```python
from build123d import *
from OCP.BRepFilletAPI import BRepFilletAPI_MakeChamfer

# Parameters (mm, degrees)
SKETCH_1_R          = 5
EXTRUDE_1_DEPTH     = 6
CUT_EXTRUDE_1_DEPTH = 3
SKETCH_3_R          = 3
EXTRUDE_2_DEPTH     = 8
CHAMFER_1_SIZE      = 0.75
FILLET_1_R          = 0.769230769
CHAMFER_2_SIZE      = 1.44092219
CHAMFER_2_SIZE2     = 2.495750443
FILLET_2_R          = 0.1


with BuildPart() as part:
    # 草图1 → 凸台-拉伸1 (new body)
    with BuildSketch(Plane.XY):
        Circle(SKETCH_1_R)
    extrude(amount=EXTRUDE_1_DEPTH)

    # 草图2 → 切除-拉伸1 (cut)
    with BuildSketch(Plane.XY.offset(6)):
        Polygon((2.5, 1.443375673), (0, 2.886751346), (-2.5, 1.443375673), (-2.5, -1.443375673), (0, -2.886751346), (2.5, -1.443375673), align=None)
    extrude(amount=-CUT_EXTRUDE_1_DEPTH, mode=Mode.SUBTRACT)

    # 草图3 → 凸台-拉伸2 (add)
    with BuildSketch(Plane(origin=(0, 0, 0), x_dir=(-1, 0, 0), z_dir=(0, 0, -1))):
        with Locations(Location((0, 0, 0), (0, 0, 180))):
            Circle(SKETCH_3_R)
    extrude(amount=EXTRUDE_2_DEPTH)

    # 倒角1
    chamfer_1_edges = [part.edges().sort_by_distance(p)[0] for p in [
        (-3, 0, -8),
    ]]
    chamfer(chamfer_1_edges, length=CHAMFER_1_SIZE)

    # 圆角1
    fillet_1_edges = [part.edges().sort_by_distance(p)[0] for p in [
        (-5, 0, 6),
    ]]
    fillet(fillet_1_edges, radius=FILLET_1_R)

    # 倒角2: one chamfer whose edges measure the first distance from different faces: ONE call of the kernel's chamfer builder (chamfer() names one face for all edges)
    chamfer_2_edges_1 = [part.edges().sort_by_distance(p)[0] for p in [
        (1.25, 2.165063509, 3),
    ]]
    chamfer_2_side_1 = [part.faces().sort_by_distance(p)[0] for p in [
        (1.25, 2.165063509, 4.5),
    ]]
    chamfer_2_edges_2 = [part.edges().sort_by_distance(p)[0] for p in [
        (2.5, 0, 3),
    ]]
    chamfer_2_side_2 = [part.faces().sort_by_distance(p)[0] for p in [
        (2.5, 0, 4.5),
    ]]
    chamfer_2_edges_3 = [part.edges().sort_by_distance(p)[0] for p in [
        (1.25, -2.165063509, 3),
    ]]
    chamfer_2_side_3 = [part.faces().sort_by_distance(p)[0] for p in [
        (1.25, -2.165063509, 4.5),
    ]]
    chamfer_2_edges_4 = [part.edges().sort_by_distance(p)[0] for p in [
        (-1.25, -2.165063509, 3),
    ]]
    chamfer_2_side_4 = [part.faces().sort_by_distance(p)[0] for p in [
        (-1.25, -2.165063509, 4.5),
    ]]
    chamfer_2_edges_5 = [part.edges().sort_by_distance(p)[0] for p in [
        (-2.5, 0, 3),
    ]]
    chamfer_2_side_5 = [part.faces().sort_by_distance(p)[0] for p in [
        (-2.5, 0, 4.5),
    ]]
    chamfer_2_edges_6 = [part.edges().sort_by_distance(p)[0] for p in [
        (-1.25, 2.165063509, 3),
    ]]
    chamfer_2_side_6 = [part.faces().sort_by_distance(p)[0] for p in [
        (-1.25, 2.165063509, 4.5),
    ]]
    chamfer_2 = BRepFilletAPI_MakeChamfer(part.part.solid().wrapped)
    for e in chamfer_2_edges_1:
        chamfer_2.Add(CHAMFER_2_SIZE, CHAMFER_2_SIZE2, e.wrapped, chamfer_2_side_1[0].wrapped)  # the first distance lies on this face
    for e in chamfer_2_edges_2:
        chamfer_2.Add(CHAMFER_2_SIZE, CHAMFER_2_SIZE2, e.wrapped, chamfer_2_side_2[0].wrapped)  # the first distance lies on this face
    for e in chamfer_2_edges_3:
        chamfer_2.Add(CHAMFER_2_SIZE, CHAMFER_2_SIZE2, e.wrapped, chamfer_2_side_3[0].wrapped)  # the first distance lies on this face
    for e in chamfer_2_edges_4:
        chamfer_2.Add(CHAMFER_2_SIZE, CHAMFER_2_SIZE2, e.wrapped, chamfer_2_side_4[0].wrapped)  # the first distance lies on this face
    for e in chamfer_2_edges_5:
        chamfer_2.Add(CHAMFER_2_SIZE, CHAMFER_2_SIZE2, e.wrapped, chamfer_2_side_5[0].wrapped)  # the first distance lies on this face
    for e in chamfer_2_edges_6:
        chamfer_2.Add(CHAMFER_2_SIZE, CHAMFER_2_SIZE2, e.wrapped, chamfer_2_side_6[0].wrapped)  # the first distance lies on this face
    add(Compound.cast(chamfer_2.Shape()), mode=Mode.REPLACE)

    # 圆角2
    fillet_2_edges = [part.edges().sort_by_distance(p)[0] for p in [
        (-3, 0, 0),
    ]]
    fillet(fillet_2_edges, radius=FILLET_2_R)


solid = part.part
```
Check sheet for the modelled part. Datum: model origin and axes. Units: mm. A direction names the side the tool comes from. Round coordinates to 2 decimals unless told otherwise and drop trailing zeros. Loops run counter-clockwise (first coordinate to the right, second up) from the corner with the lowest first, then second, coordinate; pieces in that order, holes last. Notation, with made-up numbers: M -20.75,0.25 L 26.25,0.25 A30 cw 26.25,27.25 Z; hole C 52.5,65.25 d6. An arc over 180 degrees is marked long. Answer as a JSON object with one key per item and string values.
1. Section check A-A (z = 4). Record the boundary of the cut face in (x, y), plus the area to 3 significant figures.
Reply:
{"outline": "C 0,0 d10; hole M -1.74,-1 L 0,-2 L 1.74,-1 L 1.74,1 L 0,2 L -1.74,1 Z", "area": "68.1 mm²"}
2. Mould release check, pull along X, two halves, no side actions. Record for faces 1 (the cylindrical face through (2.86, -0.9, -3.62)), 2 (the flat face through (0, 0, -8)), 3 (the flat face through (-1.233, 2.175, 5.231)): pulls with the +X half, pulls with the -X half, needs draft (parallel to the pull), parting line crosses it, or undercut.
Reply:
{"face 1": "parting line crosses it", "face 2": "needs draft", "face 3": "undercut"}
3. Gauge pin test, flat ends, axial feed: P1, Ø1, axis at y = -2.5, z = 4, coming from the +X side; P2, Ø1.5, axis at y = 2, z = -3.5, coming from the -X side; P3, Ø0.5, axis at y = -0.5, z = 5, coming from the +X side. Record the tip position at first contact, or that the pin passes through.
Reply:
{"P1": "stops at x = 4.58", "P2": "stops at x = -2.73", "P3": "stops at x = 4.99"}
4. Section check B-B (z = -6.25). Record the boundary of the cut face in (x, y).
Reply:
{"outline": "C 0,0 d6"}
5. Scan lines: line 1 (Z direction, x = 0, y = 4); line 2 (Y direction, x = -0.75, z = 4.5); line 3 (Z direction, x = -2, y = 1.5). Record each from-to range of solid material in increasing order.
Reply:
{"line 1": "z = 0 to 6", "line 2": "y = -4.94 to -2.45, 2.45 to 4.94", "line 3": "z = -7.75 to 4.32"}
6. Access from +Z, -Z, +X, -X, +Y, -Y to the whole of each face (thin tool, end or side, straight path). Record for faces 4 (the flat face through (-0.1, -3.3, 0)), 5 (the flat face through (0.74, -1.32, 3.87)), 6 (the flat face through (2, 2, 6)).
Reply:
{"face 4": "-Z", "face 5": "+Z", "face 6": "+Z, +X, -X, +Y, -Y"}
7. Section check C-C (z = 0.25). Record the boundary of the cut face in (x, y), plus the area to 3 significant figures.
Reply:
{"outline": "C 0,0 d10", "area": "78.5 mm²"}
